Study the drawing (mm; zero at the part's minimum x, y, z) and answer. A direction names the side the tool comes from. Coordinates: 2 decimals unless noted, no trailing zeros. Loops run counter-clockwise (first coordinate to the right, second up) from the corner with the lowest first, then second, coordinate; pieces in that order, holes last. Notation, with made-up numbers: (33.5, 43.5) - (43.5, 43.5) arc R6 cw to (43.5, 51.5) - close; hole circle Ø9 at (31, 36.25). An arc over 180 degrees is marked (long way). Put each result on its own line as item: value.
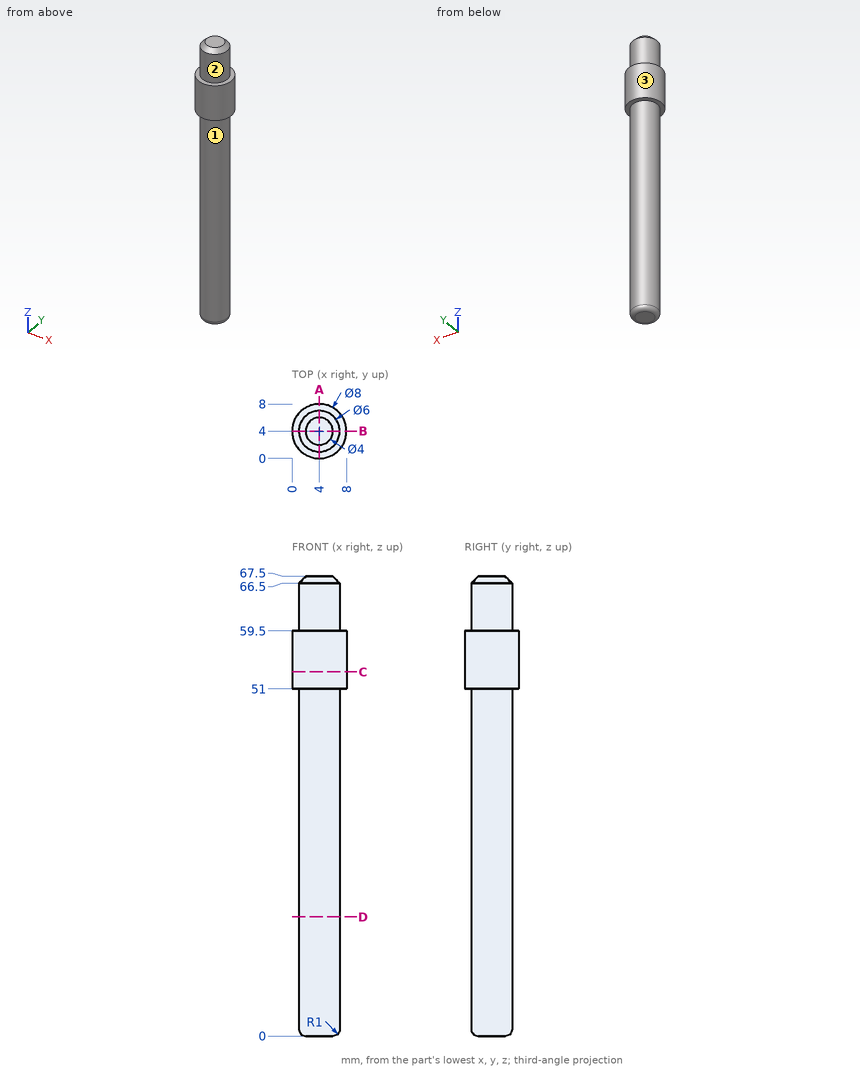
1) The part is cut by section C-C (z = 53.5). Give the vertices of the cut face in (x, y).
Found:
outline: circle Ø8 at (4, 4)
2) The part is cut by section A-A (x = 4). Give the vertices of the cut face in (y, z), and give its area (3 significant figures).
Found:
outline: (0, 51) - (1, 51) - (1, 1) arc R1 ccw to (2, 0) - (6, 0) arc R1 ccw to (7, 1) - (7, 51) - (8, 51) - (8, 59.5) - (7, 59.5) - (7, 66.5) - (6, 67.5) - (2, 67.5) - (1, 66.5) - (1, 59.5) - (0, 59.5) - close
area: 421 mm^2
3) Each of these flat-tipped pins is pushed along its axis until it touches: pin 1 (1 mm diameter, centred on y = 2.5, z = 16.5, fed in from -X); pin 2 (1 mm diameter, centred on x = 5.5, z = 57, fed in from +Y); pin 3 (4 mm diameter, centred on x = 6, z = 48.5, fed in from -Y). Where does it stop, or does it pass through?
Found:
pin 1: stops at x = 1.17
pin 2: stops at y = 7.87
pin 3: stops at y = 1
4) The part is cut by section D-D (z = 17.5). Give the vertices of the cut face in (x, y), and give its area (3 significant figures).
Found:
outline: circle Ø6 at (4, 4)
area: 28.3 mm^2
5) Straight lines are drawn through the part: L1, parallel to Z at x = 1, y = 6; L2, parallel to X at y = 4.25, z = 24.5; L3, parallel to Y at x = 6.75, z = 47.5. For each, find the intervals that lie inside material, in ascending order. Write a range as [from, to].
Found:
L1: z = [51, 59.5]
L2: x = [1.01, 6.99]
L3: y = [2.8, 5.2]
6) For the marked faces 1, 2 and 3, determine the directions among +Z, -Z, +X, -X, +Y, -Y from which every point of the face is accessible in a straight line to the end or side of a thin tool.
Found:
face 1: -Z
face 2: +Z
face 3: +Z, -Z
